Can you work these out from the model? Positions are in its coordinate system, mm. Round coordinates to 2 decimals unless told otherwise and drop trailing zeros. Loops run counter-clockwise (first coordinate to the right, second up) from the corner with the lowest first, then second, coordinate; pieces in that order, holes last. Notation, with made-up numbers: (-20, 4.25) -> (30, 4.25) arc R15 ccw to (30, 28.25) -> close; hole circle Ø10 at (-9, 46.25). An arc over 180 degrees is marked (long way). Use a Markdown table: item, result.
from build123d import *

# Parameters (mm, degrees)
SKETCH1_W           = 177.8
SKETCH1_H           = 13
BOSS_EXTRUDE1_DEPTH = 20
CHAMFER1_SIZE       = 3
SKETCH2_R           = 5
CUT_EXTRUDE1_DEPTH  = 13
LPATTERN1_COUNT     = 2
LPATTERN1_PITCH     = 157.8


with BuildPart() as part:
    # Sketch1 → Boss-Extrude1 (new body)
    with BuildSketch(Plane.XY):
        Rectangle(SKETCH1_W, SKETCH1_H)
    extrude(amount=BOSS_EXTRUDE1_DEPTH)

    # Chamfer1
    chamfer1_edges = [part.edges().sort_by_distance(p)[0] for p in [
        (-88.9, 0, 20),
        (88.9, 0, 20),
        (-88.9, 0, 0),
        (88.9, 0, 0),
    ]]
    chamfer(chamfer1_edges, length=CHAMFER1_SIZE)

    # Sketch2 → Cut-Extrude1 (cut)
    with BuildSketch(Plane(origin=(0, 6.5, 0), x_dir=(1, 0, 0), z_dir=(0, 1, 0))):
        with Locations(Location((-78.9, -10, 0), (0, 0, 180))):
            Circle(SKETCH2_R)
    cut_extrude1 = extrude(amount=-CUT_EXTRUDE1_DEPTH, mode=Mode.SUBTRACT)

    # LPattern1: Cut-Extrude1 ×2
    with Locations(*[(i * LPATTERN1_PITCH, 0, 0) for i in range(1, LPATTERN1_COUNT)]):
        add(cut_extrude1, mode=Mode.SUBTRACT)


solid = part.part
1. I want a section at A-A (z = 10). Please give me the cut outline in (x, y), plus the area to 3 significant figures.
Answer sheet:
| item | result |
|---|---|
| outline | (-88.9, -6.5) -> (-83.9, -6.5) -> (-83.9, 6.5) -> (-88.9, 6.5) -> close; (-73.9, -6.5) -> (73.9, -6.5) -> (73.9, 6.5) -> (-73.9, 6.5) -> close; (83.9, -6.5) -> (88.9, -6.5) -> (88.9, 6.5) -> (83.9, 6.5) -> close |
| area | 2,050 mm² |
2. I need wall thicknesses on line 1 (Z direction, x = -78.9, y = 2.25); line 2 (X direction, y = 3.75, z = 9.5); line 3 (X direction, y = 2.75, z = 7). Which ranges of each line are inside material? Lowest first, please.
Answer sheet:
| item | result |
|---|---|
| line 1 | z = 0 to 5, 15 to 20 |
| line 2 | x = -88.9 to -83.87, -73.93 to 73.93, 83.87 to 88.9 |
| line 3 | x = -88.9 to -82.9, -74.9 to 74.9, 82.9 to 88.9 |
3. Will this pin go through, and if not, where does the flat tip stop? pin 1 Ø2 at (y, z) = (0, 17.5) entering from -X.
Answer sheet:
| item | result |
|---|---|
| pin 1 | stops at x = -88.9 |
4. If we mould it in two halves opening along X, with no side actions, what happens to faces 1 (the flat face through (88.9, 0, 10)), 2 (the flat face through (-1, -6.5, 10)), 3 (the cylindrical face through (-73.905, 0.091, 10.22))? For each: +X half, -X half, draft (parallel to the pull), parting line (faces both ways), or undercut.
Answer sheet:
| item | result |
|---|---|
| face 1 | +X half |
| face 2 | draft |
| face 3 | undercut |
5. I want a section at B-B (x = 78.9). Please give me the cut outline in (y, z).
Answer sheet:
| item | result |
|---|---|
| outline | (-6.5, 0) -> (6.5, 0) -> (6.5, 5) -> (-6.5, 5) -> close; (-6.5, 15) -> (6.5, 15) -> (6.5, 20) -> (-6.5, 20) -> close |
6. I want a section at C-C (y = 5). Please give me the cut outline in (x, z).
Answer sheet:
| item | result |
|---|---|
| outline | (-88.9, 3) -> (-85.9, 0) -> (85.9, 0) -> (88.9, 3) -> (88.9, 17) -> (85.9, 20) -> (-85.9, 20) -> (-88.9, 17) -> close; hole circle Ø10 at (-78.9, 10); hole circle Ø10 at (78.9, 10) |
